```python
from build123d import *

# Parameters (mm, degrees)
SKETCH1_R           = 2.413
BOSS_EXTRUDE1_DEPTH = 2.413
CHAMFER1_SIZE       = 0.762


with BuildPart() as part:
    # Sketch1 → Boss-Extrude1 (new, symmetric)
    with BuildSketch(Plane(origin=(0, 0, 0), x_dir=(1, 0, 0), z_dir=(0, 1, 0))):
        with BuildLine():
            Line((-76.2, -18.7325), (76.2, -18.7325))
            ThreePointArc((76.2, -18.7325), (83.693, -11.2395), (76.2, -3.7465))
            Line((76.2, -3.7465), (31.039358608, -3.7465))
            ThreePointArc((31.039358608, -3.7465), (22.086845014, -0.981348411), (16.253078783, 6.35082279))
            ThreePointArc((16.253078783, 6.35082279), (0, 17.4498), (-16.253078783, 6.35082279))
            ThreePointArc((-16.253078783, 6.35082279), (-22.086845014, -0.981348411), (-31.039358608, -3.7465))
            Line((-31.039358608, -3.7465), (-76.2, -3.7465))
            ThreePointArc((-76.2, -3.7465), (-83.693, -11.2395), (-76.2, -18.7325))
        make_face()
        with Locations(Location((76.2, -11.2395, 0), (0, 0, 270))):
            Circle(SKETCH1_R, mode=Mode.SUBTRACT)
        with Locations(Location((-76.2, -11.2395, 0), (0, 0, 270))):
            Circle(SKETCH1_R, mode=Mode.SUBTRACT)
        with BuildLine():
            ThreePointArc((3.174972166, -8.966794468), (0, 9.5123), (-3.174972166, -8.966794468))
            ThreePointArc((-3.174972166, -8.966794468), (0, -12.1285), (3.174972166, -8.966794468))
        make_face(mode=Mode.SUBTRACT)
    extrude(amount=BOSS_EXTRUDE1_DEPTH, both=True)

    # Chamfer1
    chamfer1_edges = [part.edges().sort_by_distance(p)[0] for p in [
        (76.2, -2.413, 8.8265),
        (76.2, 2.413, 8.8265),
        (-76.2, -2.413, 8.8265),
        (-76.2, 2.413, 8.8265),
    ]]
    chamfer(chamfer1_edges, length=CHAMFER1_SIZE)


solid = part.part
```
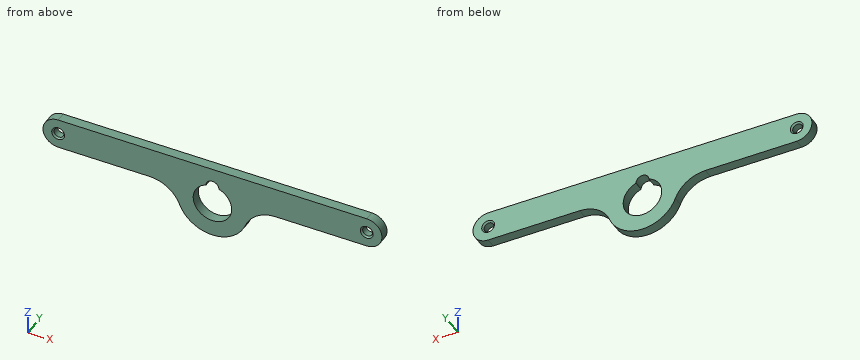
Geometry: final body of the model. Coordinates: model frame, mm. Coordinates: 2 decimals unless noted, no trailing zeros. Order: outer loops, then holes, each group sorted by start corner. A loop starts at its lowest first (then second) coordinate and runs counter-clockwise, first axis right, second up. Notation, with made-up numbers: (83, 79.25) - (98, 79.25) arc R8 cw to (98, 87.25) - close; hole circle Ø1 at (61, 50). An arc over 180 degrees is marked (long way). Return JSON: item names as keys, results as strings. Group by question number.
1. Cut plane C-C (x = 33.5). Output: boundary loops of the cut face in (y, z), plus the area to 3 significant figures.
2. Cut plane B-B (z = 0). Output: boundary loops of the cut face in (x, y).
3. Material intervals for line 1 along X through (y, z) = (1.95, 11); line 2 along X through (y, z) = (-2, 13.5); line 3 along Z through (x, y) = (0, -0.6), sorted ascending. Write a range as [from, to].
4. Cut plane A-A (y = 0.3). Count the separate pieces of the cut face and the enclosed holes in it, plus the area to 3 significant figures.
5. Cut plane D-D (z = -14). Output: boundary loops of the cut face in (x, y), plus the area to 3 significant figures.
6. Pin query (flat end, axial travel): pin 1 (7.5 mm diameter, centred on x = 76.2, z = 11.24, fed in from +Y); pin 2 (1 mm diameter, centred on x = 40.5, y = 0, fed in from -Z). Return the tip coordinate at first contact, or that it passes through.
Resolved:
{
 "1": {"outline": "(-2.41, 3.75) - (2.41, 3.75) - (2.41, 18.73) - (-2.41, 18.73) - close", "area": "72.3 mm²"},
 "2": {"outline": "(-20.8, -2.41) - (-9.51, -2.41) - (-9.51, 2.41) - (-20.8, 2.41) - close; (9.51, -2.41) - (20.8, -2.41) - (20.8, 2.41) - (9.51, 2.41) - close"},
 "3": {"line 1": "x = [-83.69, -78.9], [-73.5, -2.43], [2.43, 73.5], [78.9, 83.69]", "line 2": "x = [-83.34, -77.79], [-74.61, 74.61], [77.79, 83.34]", "line 3": "z = [-17.45, -9.51], [12.13, 18.73]"},
 "4": {"separate pieces": "1", "enclosed holes": "3", "area": "2,800 mm²"},
 "5": {"outline": "(-10.42, -2.41) - (10.42, -2.41) - (10.42, 2.41) - (-10.42, 2.41) - close", "area": "101 mm²"},
 "6": {"pin 1": "stops at y = 2.41", "pin 2": "stops at z = 3.75"}
}
